from build123d import *

# Parameters (mm, degrees)
SKETCH1_R   = 4
SKETCH1_R_2 = 3


with BuildPart() as part:
    # Sweep1: sweep along a path in Sketch2
    with BuildLine(Plane(origin=(0, 0, 0), x_dir=(0, 0, -1), z_dir=(1, 0, 0))) as sweep1_path:
        Line((0, 0), (0, 390))
        ThreePointArc((0, 390), (2.928932188, 397.071067812), (10, 400))
        Line((10, 400), (1050, 400))
    # Sketch1 → Sweep1 (sweep)
    with BuildSketch(Plane(origin=(0, 0, 0), x_dir=(1, 0, 0), z_dir=(0, 1, 0))):
        Circle(SKETCH1_R)
        Circle(SKETCH1_R_2, mode=Mode.SUBTRACT)
    sweep(path=sweep1_path.line)


solid = part.part
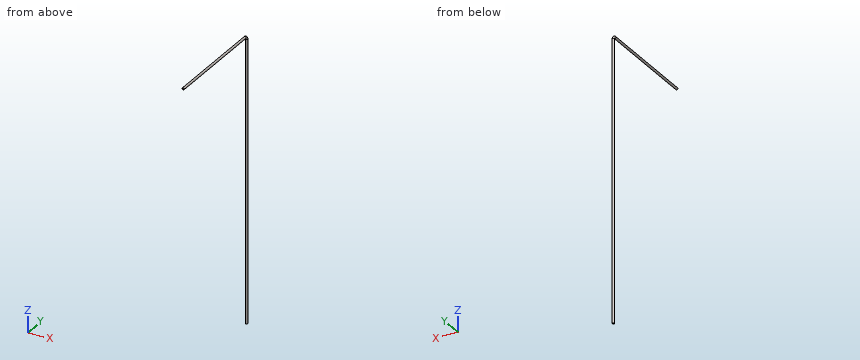
The listing builds one solid part. Answer for the finished solid, in the listing's coordinates (mm). Coordinates: 2 decimals unless noted, no trailing zeros. Write each loop counter-clockwise with the first axis right and the second up, starting at its lowest first coordinate (ties: lowest second). Pieces come first, ordered by that corner, then holes. Notation, with made-up numbers: M 18.5,41 L 43.5,41 A17 ccw 43.5,63 Z; hole C -29,25 d5. An arc over 180 degrees is marked long. Write each question's results on one line, items separated by ' | '.
Item 1: The part is cut by section C-C on z = -893. Determine the outline of the cut face in (x, y).
Answer below:
outline: C 0,400 d8; hole C 0,400 d6
Item 2: The part is cut by section A-A on x = 0. Determine the outline of the cut face in (y, z), and give its area (3 significant figures).
Answer below:
outline: M 0,-4 L 390,-4 A6 cw 396,-10 L 396,-1050 L 397,-1050 L 397,-10 A7 ccw 390,-3 L 0,-3 Z; M 0,3 L 390,3 A13 cw 403,-10 L 403,-1050 L 404,-1050 L 404,-10 A14 ccw 390,4 L 0,4 Z | area: 2,890 mm2
Item 3: The part is cut by section B-B on y = 320. Determine the outline of the cut face in (x, z), and give its area (3 significant figures).
Answer below:
outline: C 0,0 d8; hole C 0,0 d6 | area: 22.0 mm2
Item 4: Given P1, Ø3.5, axis at x = 0, z = 0, coming from the -Y side, flat-ended and moving along its own axis, determine where the tip first touches the part or whether it passes through.
Answer below:
P1: y = 395.56
Item 5: Consider probe 1 along X at (y, z) = (400, -373.5); probe 2 along Y at (x, z) = (0, -281); probe 3 along Z at (x, y) = (-1, 235.5). Determine where each line is inside the solid, lowest interval first. Write a range as [from, to].
Answer below:
probe 1: [-4, -3], [3, 4] | probe 2: [396, 397], [403, 404] | probe 3: [-3.87, -2.83], [2.83, 3.87]
